from build123d import *

# Parameters (mm, degrees)
CUT_EXTRUDE1_DEPTH = 1


with BuildPart() as part:
    # Sketch1 → Revolve1 (revolve)
    with BuildSketch(Plane.XY, mode=Mode.PRIVATE) as revolve1_sk:
        Polygon((-2, 0), (-2, 1.646666667), (-1.746666667, 1.9), (0, 1.9), (0, 1), (4.754266, 1), (5, 0.754266), (5, 0), align=None)
    revolve(revolve1_sk.sketch.rotate(Axis((5, 0, 0), (-1, 0, 0)), 270), axis=Axis((5, 0, 0), (-1, 0, 0)))

    # Sketch2 → Cut-Revolve1 (revolve, cut)
    with BuildSketch(Plane.XY, mode=Mode.PRIVATE) as cut_revolve1_sk:
        Polygon((-2, 0), (-2, 0.75), (-1, 0.75), (-0.799038106, 0), align=None)
    revolve(cut_revolve1_sk.sketch.rotate(Axis((-0.799038106, 0, 0), (-1, 0, 0)), 270), axis=Axis((-0.799038106, 0, 0), (-1, 0, 0)), mode=Mode.SUBTRACT)

    # Sketch3 → Cut-Extrude1 (cut)
    with BuildSketch(Plane(origin=(-2, 0, 0), x_dir=(0, 0, -1), z_dir=(1, 0, 0))):
        Polygon((-0.75, 0.433012702), (-0.75, -0.433012702), (0, -0.866025404), (0.75, -0.433012702), (0.75, 0.433012702), (0, 0.866025404), align=None)
    extrude(amount=CUT_EXTRUDE1_DEPTH, mode=Mode.SUBTRACT)


solid = part.part
Could you check a few things on this model? Use its own coordinates, in mm. A direction names the side the tool comes from. Give positions to 0.01 mm unless a question says otherwise; leave off trailing zeros. Write each loop counter-clockwise with the first axis right and the second up, starting at its lowest first coordinate (ties: lowest second). Pieces come first, ordered by that corner, then holes. Notation, with made-up numbers: (51, 76.5) -> (74, 76.5) arc R22 cw to (74, 91.5) -> close; hole circle Ø9 at (42, 5). An arc over 180 degrees is marked (long way). Write each question's results on one line, items separated by ' | '. Start each with the question number.
Q1. Suppose I cut it at A-A, the plane x = 4.5. List the corners of the cut face in (y, z) for me, and give its area (3 significant figures).
Q2. Which directions (+Z, -Z, +X, -X, +Y, -Y) give clear straight access to the entire face, cutting with the end or side of a thin tool? Please do faces 1 (the face through (2, -1, 0)), 2 (the face through (5, 0, 0)), 3 (the face through (-1.5, 0, -0.75)).
Q3. I'm going to push flat-ended pins straight in: pin 1 Ø1 at (x, y) = (1, 0.5) entering from -Z; pin 2 Ø2 at (x, y) = (2, -0.5) entering from +Z; pin 3 Ø2 at (y, z) = (0, 0) entering from -X. Where does each tip first touch, or does it pass through?
Q4. I need wall thicknesses on probe 1 along X at (y, z) = (0.45, -0.95); probe 2 along Y at (x, z) = (0.75, -0.5); probe 3 along Z at (x, y) = (1.5, 0.9). Which ranges of each line are inside material? Lowest first, please.
Q5. We'd pull the mould along Y, two halves only. Please class faces 4 (the face through (-1.5, 0, 0.75)), 5 (the face through (0, -1, 1)), 6 (the face through (-0.861, -0.728, 1.755)): +Y half, -Y half, draft (parallel to the pull), parting line (faces both ways), or undercut.
Outcome:
1) outline: circle Ø2 at (0, 0) | area: 3.14 mm2
2) face 1: +X | face 2: +Z, -Z, +X, +Y, -Y | face 3: -X
3) pin 1: z = -1 | pin 2: z = 1 | pin 3: x = -2
4) probe 1: -2 to 0 | probe 2: -0.87 to 0.87 | probe 3: -0.44 to 0.44
5) face 4: undercut | face 5: draft | face 6: parting line
